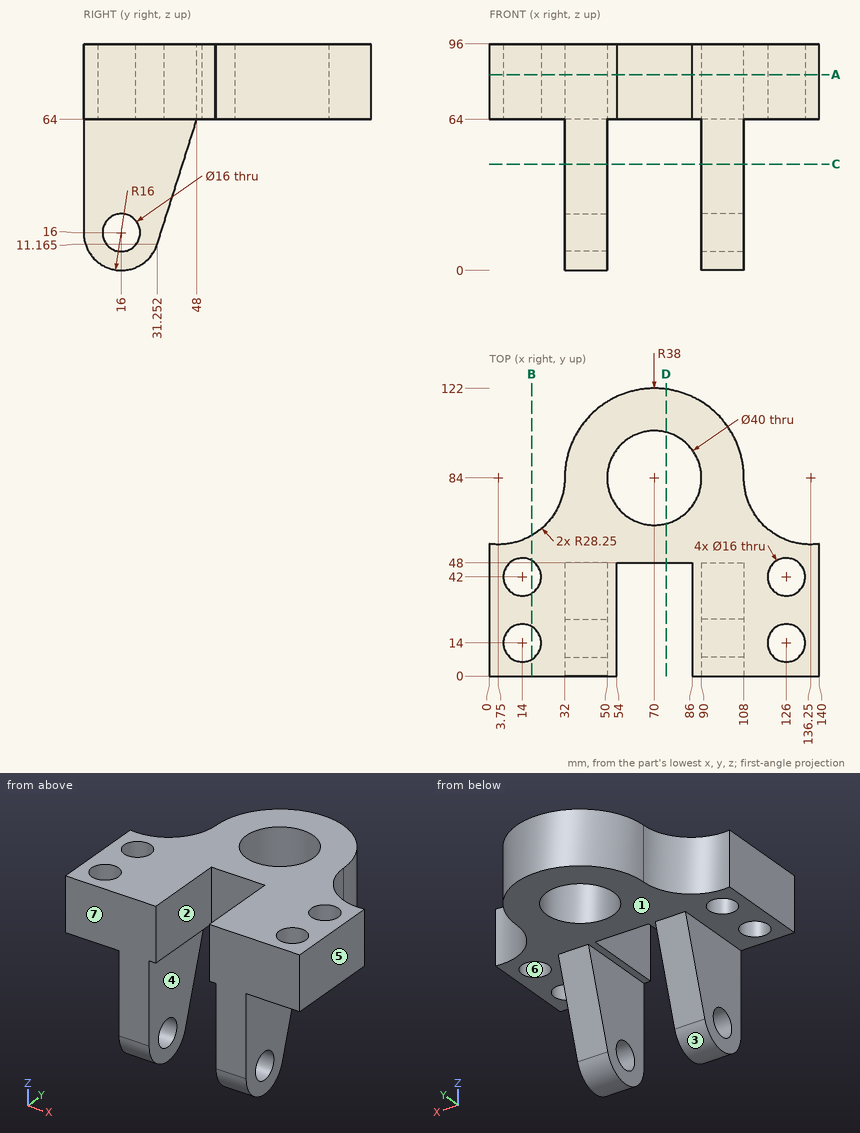
Job drawing, mm, ordinate dimensions from the low corner. One solid piece. A direction names the side the tool comes from. Round coordinates to 2 decimals unless told otherwise and drop trailing zeros. Loops run counter-clockwise (first coordinate to the right, second up) from the corner with the lowest first, then second, coordinate; pieces in that order, holes last. Notation, with made-up numbers: (-31, -0.75) -> (-10, -0.75) arc R33 ccw to (-10, 35.25) -> close; hole circle Ø5 at (-17.5, -18). An arc over 180 degrees is marked (long way). Use CSV: the item, a comma, the result in double quotes. Start each with the question number.
Q1. Saw through at B-B on x = 18. Give the cut face in (y, z), and give its area (3 significant figures).
Q2. Saw through at D-D on x = 75. Give the cut face in (y, z) (1 decimal).
Q3. Drill centre lines: L1, parallel to Y at x = 126, z = 88 (1 decimal); L2, parallel to X at y = 20, z = 71; L3, parallel to X at y = 28, z = 66. Where is each one in solid material? Low to high.
Q4. Flat gauge pins, fed straight in: pin 1 Ø10 at (y, z) = (22, 43) entering from -X; pin 2 Ø1.5 at (y, z) = (100, 79.5) entering from +X. Where does each tip first touch, or does it go through?
Q5. Saw through at A-A on z = 83. Give the cut face in (x, y), and give its area (3 significant figures).
Q6. Saw through at C-C on z = 45. Give the cut face in (x, y), and give its area (3 significant figures).
Q7. Mould opens along Y. For the marked faces 5, 6 and 7 say: +Y half, -Y half, draft (parallel to the pull), parting line (faces both ways), or undercut.
Q8. Which spindle directions (+Z, -Z, +X, -X, +Y, -Y) get a long thin tool onto all of the face, cutting with end or side? Do the marked faces 1, 2, 3 and 4. Say none if no direction does.
Solutions:
1,outline,"(0, 64) -> (7.07, 64) -> (7.07, 96) -> (0, 96) -> close; (20.93, 64) -> (35.07, 64) -> (35.07, 96) -> (20.93, 96) -> close; (48.93, 64) -> (59.61, 64) -> (59.61, 96) -> (48.93, 96) -> close"
1,area,"1,020 mm^2"
2,outline,"(48, 64) -> (64.6, 64) -> (64.6, 96) -> (48, 96) -> close; (103.4, 64) -> (121.7, 64) -> (121.7, 96) -> (103.4, 96) -> close"
3,L1,"y = 0 to 6, 22 to 34, 50 to 57.7"
3,L2,"x = 0 to 8.71, 19.29 to 54, 86 to 120.71, 131.29 to 140"
3,L3,"x = 0 to 54, 86 to 140"
4,pin 1,"stops at x = 32"
4,pin 2,"stops at x = 104.81"
5,outline,"(0, 0) -> (54, 0) -> (54, 48) -> (86, 48) -> (86, 0) -> (140, 0) -> (140, 56) arc R28.25 cw to (108, 84) arc R38 ccw to (32, 84) arc R28.25 cw to (0, 56) -> close; hole circle Ø16 at (14, 14); hole circle Ø16 at (14, 42); hole circle Ø40 at (70, 84); hole circle Ø16 at (126, 14); hole circle Ø16 at (126, 42)"
5,area,"8,970 mm^2"
6,outline,"(32, 0) -> (50, 0) -> (50, 41.98) -> (32, 41.98) -> close; (90, 0) -> (108, 0) -> (108, 41.98) -> (90, 41.98) -> close"
6,area,"1,510 mm^2"
7,face 5,"draft"
7,face 6,"undercut"
7,face 7,"-Y half"
8,face 1,"-Z, +Y"
8,face 2,"+Z, -Z, -Y"
8,face 3,"-Z, +X, -X"
8,face 4,"-Z, +Y, -Y"
